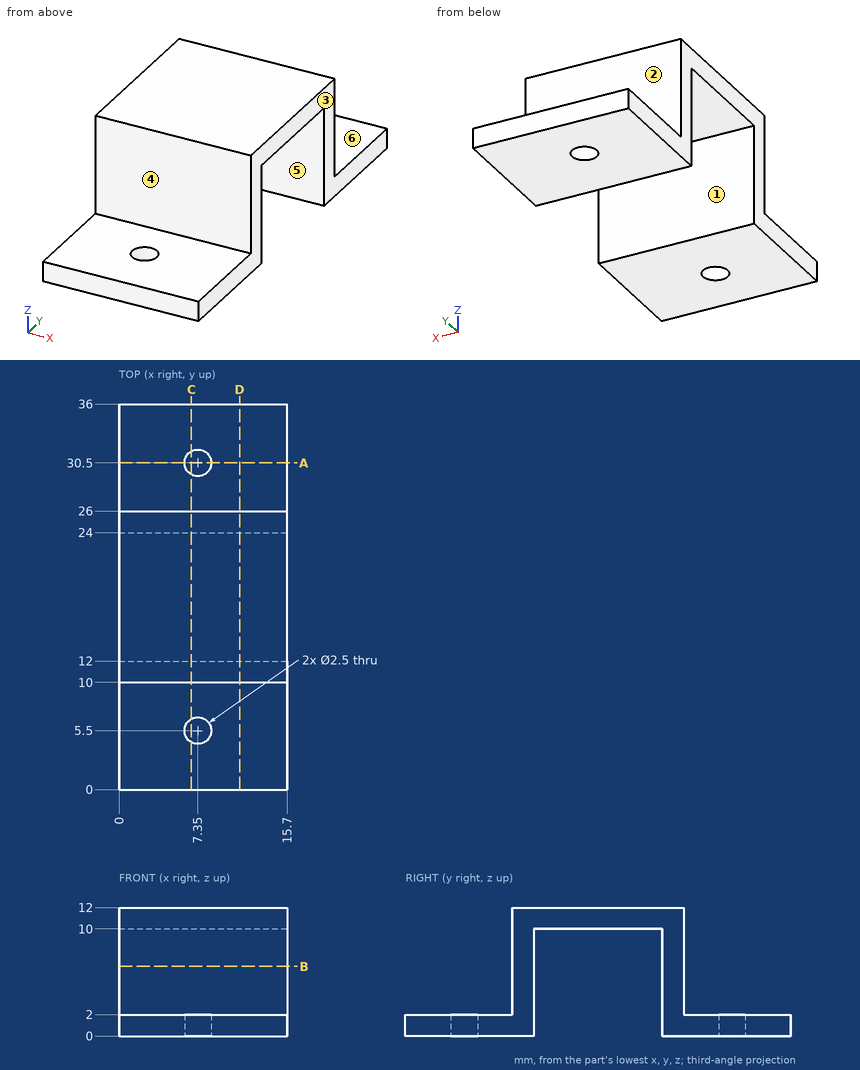
Geometry check sheet. Reference: drawing and pictorial views, mm from the part's lowest x, y, z. A direction names the side the tool comes from. Round coordinates to 2 decimals unless told otherwise and drop trailing zeros. Loops run counter-clockwise (first coordinate to the right, second up) from the corner with the lowest first, then second, coordinate; pieces in that order, holes last. Notation, with made-up numbers: M 81.25,58.5 L 132.25,58.5 A17 cw 132.25,69.5 Z; hole C -6.5,41 d2. An arc over 180 degrees is marked long. Return JSON: item names as keys, results as strings. Group by question number.
(1) Section check B-B, the plane z = 6.5. Enter the section's corners in (x, y).
(2) Mould release check, pull along Y, two halves, no side actions. Record for the marked faces 1, 2 and 3: pulls with the +Y half, pulls with the -Y half, needs draft (parallel to the pull), parting line crosses it, or undercut.
(3) Scan lines: line 1 along Y through (x, z) = (7.35, 0.45); line 2 along Y through (x, z) = (6, 3.25); line 3 along Z through (x, y) = (5.25, 26.5). Record each from-to range of solid material in increasing order. Write a range as [from, to].
(4) Go/stop test with flat-tipped pins: pin 1 (3 mm diameter, centred on x = 13, y = 21.5, fed in from -Z); pin 2 (1 mm diameter, centred on x = 2, z = 4, fed in from -Y); pin 3 (2 mm diameter, centred on x = 13.5, z = 8, fed in from +Y). Record where each tip stops, or that it passes through.
(5) Section check A-A, the plane y = 30.5. Enter the section's corners in (x, z), and give its area (3 significant figures).
(6) Set-up check for the marked faces 4, 5 and 6: record each of +Z, -Z, +X, -X, +Y, -Y from which the full face is reachable in a straight line by a thin tool's end or side.
(7) Section check D-D, the plane x = 11.25. Enter the section's corners in (y, z).
(8) Section check C-C, the plane x = 6.75. Enter the section's corners in (y, z), and give its area (3 significant figures).
Data:
{
 "1": {"outline": "M 0,10 L 15.7,10 L 15.7,12 L 0,12 Z; M 0,24 L 15.7,24 L 15.7,26 L 0,26 Z"},
 "2": {"face 1": "undercut", "face 2": "pulls with the +Y half", "face 3": "needs draft"},
 "3": {"line 1": "[0, 4.25], [6.75, 12], [24, 29.25], [31.75, 36]", "line 2": "[10, 12], [24, 26]", "line 3": "[0, 2]"},
 "4": {"pin 1": "z = 10", "pin 2": "y = 10", "pin 3": "y = 26"},
 "5": {"outline": "M 0,0 L 6.1,0 L 6.1,2 L 0,2 Z; M 8.6,0 L 15.7,0 L 15.7,2 L 8.6,2 Z", "area": "26.4 mm²"},
 "6": {"face 4": "+Z, +X, -X, -Y", "face 5": "-Z, +X, -X", "face 6": "+Z, +X, -X, +Y"},
 "7": {"outline": "M 0,0 L 12,0 L 12,10 L 24,10 L 24,0 L 36,0 L 36,2 L 26,2 L 26,12 L 10,12 L 10,2 L 0,2 Z"},
 "8": {"outline": "M 0,0 L 4.4,0 L 4.4,2 L 0,2 Z; M 6.6,0 L 12,0 L 12,10 L 24,10 L 24,0 L 29.4,0 L 29.4,2 L 26,2 L 26,12 L 10,12 L 10,2 L 6.6,2 Z; M 31.6,0 L 36,0 L 36,2 L 31.6,2 Z", "area": "103 mm²"}
}
